Part model, mm, in its own coordinate system. Round coordinates to 2 decimals unless told otherwise and drop trailing zeros. Loops run counter-clockwise (first coordinate to the right, second up) from the corner with the lowest first, then second, coordinate; pieces in that order, holes last. Notation, with made-up numbers: (81.5, -23) - (92.5, -23) arc R27 ccw to (92.5, 9) - close; hole circle Ø10 at (58.5, -30). An arc over 180 degrees is marked (long way). Put each result on its own line as item: value.
from build123d import *

# Parameters (mm, degrees)
SKETCH1_R                  = 75
BOSS_EXTRUDE1_DEPTH        = 12
F_16_0_16_DIAMETER_HOLE1_D = 16
F_30_DIAMETER_HOLE2_D      = 30


with BuildPart() as part:
    # Sketch1 → Boss-Extrude1 (new body)
    with BuildSketch(Plane(origin=(0, 0, 0), x_dir=(1, 0, 0), z_dir=(0, 1, 0))):
        with BuildLine():
            Line((225, -235), (-225, -235))
            ThreePointArc((-225, -235), (-232.071067812, -232.071067812), (-235, -225))
            Line((-235, -225), (-235, 225))
            ThreePointArc((-235, 225), (-232.071067812, 232.071067812), (-225, 235))
            Line((-225, 235), (225, 235))
            ThreePointArc((225, 235), (232.071067812, 232.071067812), (235, 225))
            Line((235, 225), (235, -225))
            ThreePointArc((235, -225), (232.071067812, -232.071067812), (225, -235))
        make_face()
        with Locations(Location((0, 0, 0), (0, 0, 270))):
            Circle(SKETCH1_R, mode=Mode.SUBTRACT)
    extrude(amount=BOSS_EXTRUDE1_DEPTH)

    # Ø16.0 (16) Diameter Hole1 (through all)
    with Locations(Plane(origin=(0, 12, 0), x_dir=(1, 0, 0), z_dir=(0, 1, 0))):
        with Locations((0, 164), (56.091303505, 154.109589809), (105.417167989, 125.631288672), (142.028166221, 82), (161.508471494, 28.478301137), (161.508471494, -28.478301137), (142.028166221, -82), (105.417167989, -125.631288672), (56.091303505, -154.109589809), (0, -164), (-56.091303505, -154.109589809), (-105.417167989, -125.631288672), (-142.028166221, -82), (-161.508471494, -28.478301137), (-161.508471494, 28.478301137), (-142.028166221, 82), (-105.417167989, 125.631288672), (-56.091303505, 154.109589809)):
            Hole(F_16_0_16_DIAMETER_HOLE1_D / 2)

    # Ø30 Diameter Hole2 (through all)
    with Locations(Plane(origin=(0, 12, 0), x_dir=(1, 0, 0), z_dir=(0, 1, 0))):
        with Locations((0, 116), (116, 0), (0, -116), (-116, 0)):
            Hole(F_30_DIAMETER_HOLE2_D / 2)


solid = part.part
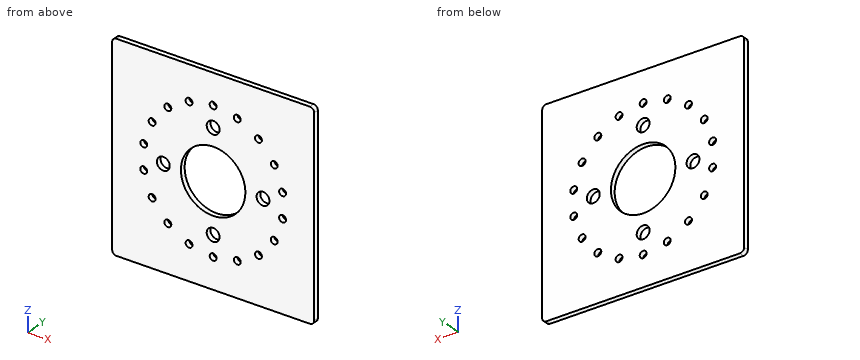
1. Band-saw the part on B-B (x = 0). List the corners of the cut face in (y, z), plus the area to 3 significant figures.
A:
outline: (0, -235) - (12, -235) - (12, -172) - (0, -172) - close; (0, -156) - (12, -156) - (12, -131) - (0, -131) - close; (0, -101) - (12, -101) - (12, -75) - (0, -75) - close; (0, 75) - (12, 75) - (12, 101) - (0, 101) - close; (0, 131) - (12, 131) - (12, 156) - (0, 156) - close; (0, 172) - (12, 172) - (12, 235) - (0, 235) - close
area: 2,740 mm²
2. Band-saw the part on A-A (z = 0). List the corners of the cut face in (x, y).
A:
outline: (-235, 0) - (-131, 0) - (-131, 12) - (-235, 12) - close; (-101, 0) - (-75, 0) - (-75, 12) - (-101, 12) - close; (75, 0) - (101, 0) - (101, 12) - (75, 12) - close; (131, 0) - (235, 0) - (235, 12) - (131, 12) - close
3. Band-saw the part on D-D (x = -159). List the corners of the cut face in (y, z), plus the area to 3 significant figures.
A:
outline: (0, -235) - (12, -235) - (12, -36.07) - (0, -36.07) - close; (0, -20.88) - (12, -20.88) - (12, 20.88) - (0, 20.88) - close; (0, 36.07) - (12, 36.07) - (12, 235) - (0, 235) - close
area: 5,280 mm²
4. Band-saw the part on C-C (y = 3.75). Give the number of separate pieces and of enclosed holes in the cut face, plus the area to 3 significant figures.
A:
separate pieces: 1
enclosed holes: 23
area: 197,000 mm²
5. Probe line 1 along X through (y, z) = (3.75, 81); line 2 along X through (y, z) = (1.75, 164); line 3 along X through (y, z) = (9.75, -79). List the from-to ranges inside material, lowest first. Write a range as [from, to].
A:
line 1: x = [-235, -149.97], [-134.09, 134.09], [149.97, 235]
line 2: x = [-235, -8], [8, 235]
line 3: x = [-235, -149.44], [-134.61, 134.61], [149.44, 235]
